For this review, use the dimensioned drawing (mm, ordinates from the lowest corner) and the shaded views. A direction names the side the tool comes from. Coordinates: 2 decimals unless noted, no trailing zeros. Write each loop counter-clockwise with the first axis right and the second up, starting at its lowest first coordinate (ties: lowest second). Pieces come first, ordered by that corner, then holes.
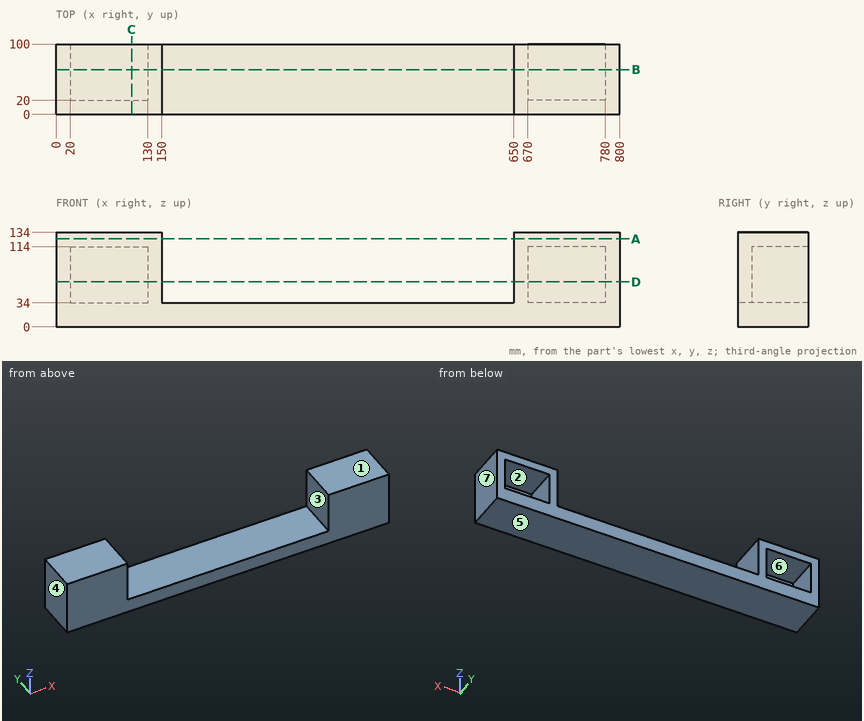
(1) Consider section D-D (z = 64). Give the boundary of the cut face in (x, y).
(2) Consider section B-B (y = 63.5). Give the boundary of the cut face in (x, z), plus the area to 3 significant figures.
(3) Consider section A-A (z = 125). Give the boundary of the cut face in (x, y).
(4) Wall thickness on line 1 (X direction, y = 86, z = 47.5); line 2 (Z direction, x = 744.5, y = 36); line 3 (X direction, y = 11.5, z = 65): over which ranges is each line inside the solid? List them lowest first.
(5) Mouldability with a two-part tool opening along X and no side actions: class the marked faces 4, 5, 6 and 7 as +X half, -X half, draft (parallel to the pull), parting line (faces both ways), or undercut.
(6) Consider section C-C (x = 107.5). Give the boundary of the cut face in (y, z).
(7) For the marked faces 1, 2 and 3, list the 3-axis set-ups (+Z, -Z, +X, -X, +Y, -Y) from which the entire face can be reached by the end or side of a thin tool; tool diameter is ignored.
(8) Insertion check: pin 1 Ø1 at (x, y) = (449, 60.5) entering from +Z; pin 2 Ø4 at (x, z) = (215, 17) entering from -Y; pin 3 Ø24 at (x, z) = (59.5, 86) entering from +Y. Each pin has a flat end and moves straight along its axis. Give the tip position at first contact, or say it passes through.
Results:
1. outline: (0, 0) - (150, 0) - (150, 100) - (130, 100) - (130, 20) - (20, 20) - (20, 100) - (0, 100) - close; (650, 0) - (800, 0) - (800, 100) - (780, 100) - (780, 20) - (670, 20) - (670, 100) - (650, 100) - close
2. outline: (0, 0) - (800, 0) - (800, 134) - (650, 134) - (650, 34) - (150, 34) - (150, 134) - (0, 134) - close; hole (20, 34) - (130, 34) - (130, 114) - (20, 114) - close; hole (670, 34) - (780, 34) - (780, 114) - (670, 114) - close
2. area: 39,600 mm2
3. outline: (0, 0) - (150, 0) - (150, 100) - (0, 100) - close; (650, 0) - (800, 0) - (800, 100) - (650, 100) - close
4. line 1: x = 0 to 20, 130 to 150, 650 to 670, 780 to 800
4. line 2: z = 0 to 34, 114 to 134
4. line 3: x = 0 to 150, 650 to 800
5. face 4: -X half
5. face 5: draft
5. face 6: undercut
5. face 7: +X half
6. outline: (0, 0) - (100, 0) - (100, 34) - (20, 34) - (20, 114) - (100, 114) - (100, 134) - (0, 134) - close
7. face 1: +Z, +X, -X, +Y, -Y
7. face 2: +Y
7. face 3: +Z, +Y, -Y
8. pin 1: stops at z = 34
8. pin 2: stops at y = 0
8. pin 3: stops at y = 20
